```python
from build123d import *

# Parameters (mm, degrees)
EXTRUDE_1_DEPTH     = 674
CUT_EXTRUDE_1_DEPTH = 696.773670097


with BuildPart() as part:
    # 草图1 → 凸台-拉伸1 (new, symmetric)
    with BuildSketch(Plane.XY):
        Polygon((0, 0), (65, 0), (65, 4), (8.5, 8), (8.5, 152), (65, 156), (65, 160), (0, 160), align=None)
    extrude(amount=EXTRUDE_1_DEPTH, both=True)

    # 草图4 → 切除-拉伸1 (cut, through all)
    with BuildSketch(Plane.ZY):
        Polygon((-674, 160), (-617, 160), (-617, 152), (-674, 146), align=None)
        Polygon((674, 146), (674, 160), (617, 160), (617, 152), align=None)
        Polygon((674, 0), (617, 0), (617, 8), (674, 14), align=None)
        Polygon((-674, 14), (-674, 0), (-617, 0), (-617, 8), align=None)
    extrude(amount=-CUT_EXTRUDE_1_DEPTH, mode=Mode.SUBTRACT)


solid = part.part
```
Geometry check sheet. Reference: the model listing, model coordinates, mm. Give positions to 0.01 mm unless a question says otherwise; leave off trailing zeros. Order: outer loops, then holes, each group sorted by start corner. A loop starts at its lowest first (then second) coordinate and runs counter-clockwise, first axis right, second up.
1. Section check A-A, the plane z = -307.5. Enter the section's corners in (x, y).
2. Section check B-B, the plane x = 39. Enter the section's corners in (y, z).
3. Section check C-C, the plane y = 116.5. Enter the section's corners in (x, z), and give its area (3 significant figures).
4. Thickness scan on L1, parallel to X at y = 124.5, z = -552.5; L2, parallel to Y at x = 33.5, z = 349; L3, parallel to Y at x = 11, z = -310. Record the ranges inside material, lowest first.
5. Gauge pin test, flat ends, axial feed: pin 1 Ø8 at (y, z) = (82, -27) entering from +X; pin 2 Ø6 at (y, z) = (119, -57.5) entering from -X; pin 3 Ø9 at (x, y) = (24.5, 2.5) entering from -Z; pin 4 Ø4 at (x, y) = (36.5, 5) entering from +Z. Record the tip position at first contact, or that the pin passes through.
6. Release check for a two-part mould opening along Y. For faces 1 (the face through (0, 81, 9)), 2 (the face through (33, 160, 9)), 3 (the face through (32, 0, 9)), 4 (the face through (37.15, 5.97, 8.64)) record: pulls with the +Y half, pulls with the -Y half, needs draft (parallel to the pull), parting line crosses it, or undercut.
Values follow:
1. outline: (0, 0) - (65, 0) - (65, 4) - (8.5, 8) - (8.5, 152) - (65, 156) - (65, 160) - (0, 160) - close
2. outline: (0, -617) - (5.84, -617) - (5.84, 617) - (0, 617) - close; (154.16, -617) - (160, -617) - (160, 617) - (154.16, 617) - close
3. outline: (0, -674) - (8.5, -674) - (8.5, 674) - (0, 674) - close
3. area: 11,500 mm2
4. L1: x = 0 to 8.5
4. L2: y = 0 to 6.23, 153.77 to 160
4. L3: y = 0 to 7.82, 152.18 to 160
5. pin 1: stops at x = 8.5
5. pin 2: stops at x = 0
5. pin 3: stops at z = -617
5. pin 4: stops at z = 617
6. face 1: needs draft
6. face 2: pulls with the +Y half
6. face 3: pulls with the -Y half
6. face 4: undercut
